Check sheet for the drawn part. Datum: minimum x, y, z corner. Units: mm. A direction names the side the tool comes from. Round coordinates to 2 decimals unless told otherwise and drop trailing zeros. Write each loop counter-clockwise with the first axis right and the second up, starting at its lowest first coordinate (ties: lowest second). Pieces come first, ordered by that corner, then holes. Notation, with made-up numbers: (74, 76) - (107, 76) arc R15 ccw to (107, 83) - close; hole circle Ø5 at (63, -32.75). An arc over 180 degrees is marked (long way). Write each question's results on one line, items separated by ' | '.
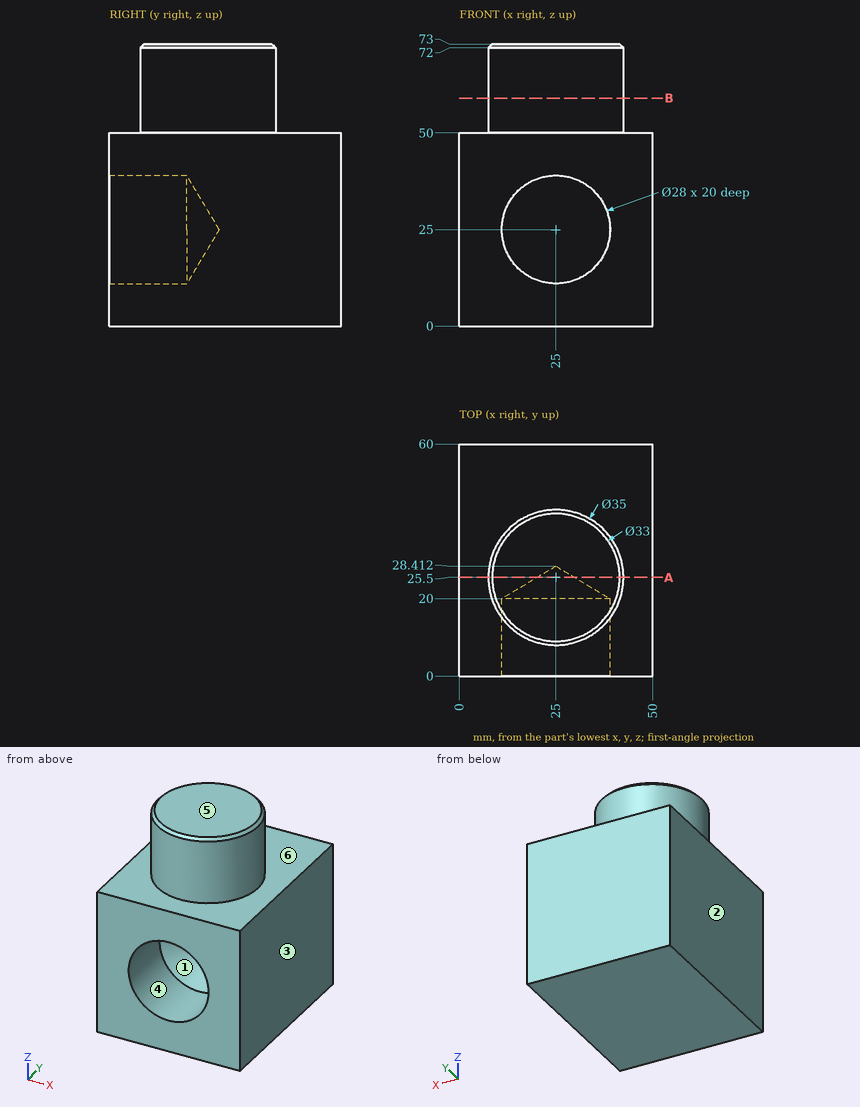
(1) Section check A-A (y = 25.5). Record the cut outline in (x, z).
Answer:
outline: (0, 0) - (50, 0) - (50, 50) - (42.5, 50) - (42.5, 72) - (41.5, 73) - (8.5, 73) - (7.5, 72) - (7.5, 50) - (0, 50) - close; hole circle Ø9.69 at (25, 25)
(2) Thickness scan on L1, parallel to Z at x = 25, y = 7; L2, parallel to Z at x = 25, y = 10.75; L3, parallel to Z at x = 7, y = 56. Record the ranges inside material, lowest first.
Answer:
L1: 0 to 11, 39 to 50 | L2: 0 to 11, 39 to 73 | L3: 0 to 50
(3) Set-up check for the marked faces 5 and 6: record each of +Z, -Z, +X, -X, +Y, -Y from which the full face is reachable in a straight line by a thin tool's end or side.
Answer:
face 5: +Z, +X, -X, +Y, -Y | face 6: +Z
(4) Section check B-B (z = 59). Record the cut outline in (x, y).
Answer:
outline: circle Ø35 at (25, 25.5)
(5) Go/stop test with flat-tipped pins: pin 1 Ø1 at (x, y) = (10.5, 21) entering from -Z; pin 2 Ø22.5 at (x, z) = (25, 25) entering from -Y; pin 3 Ø1 at (x, z) = (41.5, 55) entering from +Y; pin 4 Ø3 at (x, z) = (31.5, 32) entering from -Y. Record where each tip stops, or that it passes through.
Answer:
pin 1: z = 0 | pin 2: y = 21.65 | pin 3: y = 32.59 | pin 4: y = 21.77
(6) Mould release check, pull along X, two halves, no side actions. Record for the marked faces 1, 2, 3 and 4: released by +X, released by -X, zero draft, split by the parting line, or undercut.
Answer:
face 1: undercut | face 2: released by -X | face 3: released by +X | face 4: undercut
